For this review, take the finished solid that the model builds, in its own axes (mm). A direction names the side the tool comes from. Give positions to 0.01 mm unless a question says otherwise; leave off trailing zeros. Order: outer loops, then holes, each group sorted by start corner. A loop starts at its lowest first (then second) coordinate and runs counter-clockwise, first axis right, second up.
from build123d import *

# Parameters (mm, degrees)
SKETCH1_R                                           = 17.5
BOSS_EXTRUDE1_DEPTH                                 = 10
CHAMFER1_SIZE                                       = 0.5
HOLE_SIZE_PER_SOCKET_FLAT_COUNTEBLZKK_H_D           = 9
HOLE_SIZE_PER_SOCKET_FLAT_COUNTEBLZKK_H_CSINK_D     = 17
HOLE_SIZE_PER_SOCKET_FLAT_COUNTEBLZKK_H_CSINK_ANGLE = 90
SKETCH5_R                                           = 10
CUT_EXTRUDE1_DEPTH                                  = 4
CHAMFER2_SIZE                                       = 0.5


with BuildPart() as part:
    # Sketch1 → Boss-Extrude1 (new body)
    with BuildSketch(Plane.XY):
        Circle(SKETCH1_R)
    extrude(amount=BOSS_EXTRUDE1_DEPTH)

    # Chamfer1
    chamfer1_edges = [part.edges().sort_by_distance(p)[0] for p in [
        (-17.5, 0, 0),
        (-17.5, 0, 10),
    ]]
    chamfer(chamfer1_edges, length=CHAMFER1_SIZE)

    # Hole size (per socket flat counteBLZKk head screw type)1 (through all)
    with Locations(Plane(origin=(0, 0, 0), x_dir=(1, 0, 0), z_dir=(0, 0, -1))):
        with Locations((0, 0)):
            CounterSinkHole(HOLE_SIZE_PER_SOCKET_FLAT_COUNTEBLZKK_H_D / 2, HOLE_SIZE_PER_SOCKET_FLAT_COUNTEBLZKK_H_CSINK_D / 2, counter_sink_angle=HOLE_SIZE_PER_SOCKET_FLAT_COUNTEBLZKK_H_CSINK_ANGLE)

    # Sketch5 → Cut-Extrude1 (cut)
    with BuildSketch(Plane.XY.offset(10)):
        Circle(SKETCH5_R)
    extrude(amount=-CUT_EXTRUDE1_DEPTH, mode=Mode.SUBTRACT)

    # Chamfer2
    chamfer2_edges = [part.edges().sort_by_distance(p)[0] for p in [
        (-10, 0, 10),
    ]]
    chamfer(chamfer2_edges, length=CHAMFER2_SIZE)


solid = part.part
1) Draft analysis for pull direction X (two halves, no side actions). For faces 3 (the face through (4.3, -2.1, 6)), 4 (the face through (4, 8, 0)), 5 (the face through (-13.887, -10.648, 4.937)), state which applies: +X half, -X half, draft (parallel to the pull), parting line (faces both ways), or undercut.
Answer sheet:
face 3: undercut
face 4: draft
face 5: parting line
2) We need section A-A on y = 0. Give the boundary of the cut face in (x, z).
Answer sheet:
outline: (-17.5, 0.5) - (-17, 0) - (-8.5, 0) - (-4.5, 4) - (-4.5, 6) - (-10, 6) - (-10, 9.5) - (-10.5, 10) - (-17, 10) - (-17.5, 9.5) - close; (4.5, 4) - (8.5, 0) - (17, 0) - (17.5, 0.5) - (17.5, 9.5) - (17, 10) - (10.5, 10) - (10, 9.5) - (10, 6) - (4.5, 6) - close
3) Clearance check with flat-ended pins moving along their axes: pin 1 (4 mm diameter, centred on y = 9.5, z = 2, fed in from +X); pin 2 (5 mm diameter, centred on x = -8.5, y = -6, fed in from +Z); pin 3 (4 mm diameter, centred on x = -5, z = 3, fed in from +Y); pin 4 (16 mm diameter, centred on x = 0, y = 0, fed in from +Z). State where each tip first meets the part, or that it passes through.
Answer sheet:
pin 1: stops at x = 15.81
pin 2: stops at z = 10
pin 3: stops at y = 17.24
pin 4: stops at z = 6
4) We need section D-D on z = 1.25. Give the boundary of the cut face in (x, y).
Answer sheet:
outline: circle Ø35 at (0, 0); hole circle Ø14.5 at (0, 0)
5) To check wall thickness, follow line 1 (Y direction, x = 0, z = 8.65); line 2 (X direction, y = -8, z = 6.25); line 3 (Z direction, x = -8.5, y = 1). State the ranges of each line that lie inside material, in increasing order.
Answer sheet:
line 1: y = -17.5 to -10, 10 to 17.5
line 2: x = -15.56 to -6, 6 to 15.56
line 3: z = 0 to 6
6) We need section C-C on z = 7. Give the boundary of the cut face in (x, y).
Answer sheet:
outline: circle Ø35 at (0, 0); hole circle Ø20 at (0, 0)
7) Tool access review of faces 1 (the face through (7.3, 7.8, 10)), 2 (the face through (-2.17, -9.76, 7.77)): name each direction out of +Z, -Z, +X, -X, +Y, -Y from which nothing blocks a thin tool from reaching the whole face with its end or side.
Answer sheet:
face 1: +Z, +X, -X, +Y, -Y
face 2: +Z
